Read the model definition and answer for the solid it produces. Units are mm, in the model's axes. A direction names the side the tool comes from. Give positions to 0.01 mm unless a question says otherwise; leave off trailing zeros. Order: outer loops, then holes, each group sorted by start corner. A loop starts at its lowest first (then second) coordinate and runs counter-clockwise, first axis right, second up. Notation, with made-up numbers: (8.25, -31.5) -> (23.25, -31.5) arc R24 ccw to (23.25, -2.5) -> close; hole circle Ø6 at (-0.5, -34). An arc over 180 degrees is marked (long way). One line per question, with ' | ' between items. Start each with the question number.
```python
from build123d import *

# Parameters (mm, degrees)
SKETCH1_R           = 10
BOSS_EXTRUDE1_DEPTH = 11
CUT_EXTRUDE1_DEPTH  = 2.5
CUT_EXTRUDE2_DEPTH  = 2.5
SKETCH4_W           = 15.449608091
SKETCH4_H           = 8
CUT_EXTRUDE3_DEPTH  = 3
FILLET1_R           = 1
CUT_EXTRUDE5_START  = -1.5
CUT_EXTRUDE5_DEPTH  = 1.5


with BuildPart() as part:
    # Sketch1 → Boss-Extrude1 (new, symmetric)
    with BuildSketch(Plane.XY):
        with BuildLine():
            ThreePointArc((16.711932938, -6.452050085), (11, 0), (16.711932938, 6.452050085))
            ThreePointArc((16.711932938, 6.452050085), (0, 36), (-16.711932938, 6.452050085))
            ThreePointArc((-16.711932938, 6.452050085), (-11, 0), (-16.711932938, -6.452050085))
            ThreePointArc((-16.711932938, -6.452050085), (0, -36), (16.711932938, -6.452050085))
        make_face()
        with Locations((0, -16.5)):
            Circle(SKETCH1_R, mode=Mode.SUBTRACT)
        with Locations((0, 16.5)):
            Circle(SKETCH1_R, mode=Mode.SUBTRACT)
    extrude(amount=BOSS_EXTRUDE1_DEPTH, both=True)

    # Sketch2 → Cut-Extrude1 (cut)
    with BuildSketch(Plane.XY.offset(11)):
        with BuildLine():
            Line((-19.068213964, 20.580835235), (-15.186057607, 18.339471217))
            ThreePointArc((-15.186057607, 18.339471217), (-13.000189211, 18.186313351), (-11.533289054, 19.814097705))
            ThreePointArc((-11.533289054, 19.814097705), (9.5856448, 23.719100621), (0, 4.5))
            ThreePointArc((0, 4.5), (-4.5, 0), (0, -4.5))
            ThreePointArc((0, -4.5), (9.5856448, -23.719100621), (-11.533289054, -19.814097705))
            ThreePointArc((-11.533289054, -19.814097705), (-13.000189211, -18.186313351), (-15.186057607, -18.339471217))
            Line((-15.186057607, -18.339471217), (-19.068213964, -20.580835235))
            ThreePointArc((-19.068213964, -20.580835235), (-18.199948236, -23.500848821), (-16.887495374, -26.25))
            Line((-16.887495374, -26.25), (-14.696938457, -24.985281374))
            ThreePointArc((-14.696938457, -24.985281374), (-13.966653368, -24.87818357), (-13.36182443, -25.301229909))
            ThreePointArc((-13.36182443, -25.301229909), (14.085802756, -24.088818138), (0, -0.5))
            ThreePointArc((0, -0.5), (-0.5, 0), (0, 0.5))
            ThreePointArc((0, 0.5), (14.085802756, 24.088818138), (-13.36182443, 25.301229909))
            ThreePointArc((-13.36182443, 25.301229909), (-13.966653368, 24.87818357), (-14.696938457, 24.985281374))
            Line((-14.696938457, 24.985281374), (-16.887495374, 26.25))
            ThreePointArc((-16.887495374, 26.25), (-18.199948236, 23.500848821), (-19.068213964, 20.580835235))
        make_face()
    extrude(amount=-CUT_EXTRUDE1_DEPTH, mode=Mode.SUBTRACT)

    # Sketch3 → Cut-Extrude2 (cut)
    with BuildSketch(Plane.XY.offset(11)):
        Polygon((-17.173443463, 0.521044654), (1.285575219, -14.967911114), (-1.285575219, -18.032088886), (-19.744593902, -2.543133118), align=None)
    cut_extrude2 = extrude(amount=-CUT_EXTRUDE2_DEPTH, mode=Mode.SUBTRACT)

    # Mirror1: Cut-Extrude2 across plane
    add(cut_extrude2.mirror(Plane.ZX), mode=Mode.SUBTRACT)

    # Sketch4 → Cut-Extrude3 (cut)
    with BuildSketch(Plane(origin=(0, 0, -11), x_dir=(-1, 0, 0), z_dir=(0, 0, -1))):
        with Locations((11.224804046, 0)):
            Rectangle(SKETCH4_W, SKETCH4_H)
        with Locations((-11.224804046, 0)):
            Rectangle(SKETCH4_W, SKETCH4_H)
    extrude(amount=-CUT_EXTRUDE3_DEPTH, mode=Mode.SUBTRACT)

    # Fillet1
    fillet1_edges = [part.edges().sort_by_distance(p)[0] for p in [
        (-3.5, 4, -9.5),
        (-3.5, -4, -9.5),
        (3.5, -4, -9.5),
        (3.5, 4, -9.5),
    ]]
    fillet(fillet1_edges, radius=FILLET1_R)

    # Sketch5 → Cut-Extrude5 (cut)
    with BuildSketch(Plane(origin=(0, 0, -11), x_dir=(-1, 0, 0), z_dir=(0, 0, -1)).offset(CUT_EXTRUDE5_START)):
        with BuildLine():
            ThreePointArc((12.376524617, 4), (13.243803843, 4.912717605), (14.270776222, 5.641109269))
            Line((14.270776222, 5.641109269), (7.397387325, 9.771057976))
            ThreePointArc((7.397387325, 9.771057976), (5.606135542, 8.219224415), (3.5, 7.132503002))
            Line((3.5, 7.132503002), (3.5, 3))
            ThreePointArc((3.5, 3), (3.792893219, 3.707106781), (4.5, 4))
            Line((4.5, 4), (12.376524617, 4))
        make_face()
        with BuildLine():
            Line((7.397387325, -9.771057976), (14.270776222, -5.641109269))
            ThreePointArc((14.270776222, -5.641109269), (13.243803843, -4.912717605), (12.376524617, -4))
            Line((12.376524617, -4), (4.5, -4))
            ThreePointArc((4.5, -4), (3.792893219, -3.707106781), (3.5, -3))
            Line((3.5, -3), (3.5, -7.132503002))
            ThreePointArc((3.5, -7.132503002), (5.606135542, -8.219224415), (7.397387325, -9.771057976))
        make_face()
    extrude(amount=CUT_EXTRUDE5_DEPTH, mode=Mode.SUBTRACT)


solid = part.part
```
Q1. A cutting plane is placed at B-B, the plane x = 8. Give the number of separate pieces and of enclosed holes in the cut face, then the cut area to 3 significant figures.
Q2. Which of the six approach directions +Z, -Z, +X, -X, +Y, -Y give full straight-line access (tool end or side, diameter ignored) to faces 1 (the flat face through (-15.81, -25.63, 9.77)), 2 (the flat face through (-17.1, -19.444, 9.768)), 3 (the flat face through (-10.88, 7.68, -10.24)), 4 (the flat face through (8, -4, -10)), 5 (the flat face through (-8, 4, -9))?
Q3. A cutting plane is placed at A-A, the plane y = -16.5. Determine the outline of the cut face in (x, z).
Q4. Given P1, Ø4, axis at x = 9.5, y = -1.5, coming from the -Z side; P2, Ø1.6, axis at x = -8.5, z = -8.5, coming from the -Y side; P3, Ø8, axis at y = 9, z = -5.5, coming from the -X side; P4, Ø18, axis at x = 0, y = -16.5, coming from the -Z side, each flat-ended and moving along its own axis, determine where each tip first touches the part or whether it passes through.
Q5. A cutting plane is placed at C-C, the plane z = 1.5. Determine the outline of the cut face in (x, y), then the cut area to 3 significant figures.
Q6. A cutting plane is placed at D-D, the plane x = 15. Determine the outline of the cut face in (y, z).
Q7. Find the intervals of material crossed by line 1 (X direction, y = -16.5, z = 9.95); line 2 (Y direction, x = 0, z = 2.75); line 3 (X direction, y = 17, z = 7.75), in increasing order.
Q8. Determine the mould class of faces 6 (the flat face through (-17.2, 19.5, 9.8)), 7 (the flat face through (-15.78, 25.61, 9.77)), 8 (the flat face through (-12.06, 8.99, 9.77)), 9 (the flat face through (8, 0, -8)) for opening direction X: pulls with the +X half, pulls with the -X half, needs draft (parallel to the pull), parting line crosses it, or undercut.
Geometry results:
1) separate pieces: 3 | enclosed holes: 0 | area: 907 mm²
2) face 1: +Z, -X | face 2: +Z | face 3: -Z | face 4: -Z, +X | face 5: -Z, -X
3) outline: (-19.5, -11) -> (-10, -11) -> (-10, 11) -> (-19.5, 11) -> close; (10, -11) -> (19.5, -11) -> (19.5, 11) -> (16, 11) -> (16, 8.5) -> (12, 8.5) -> (12, 11) -> (10, 11) -> close
4) P1: z = -8 | P2: y = -34.42 | P3: x = -19.18 | P4: through
5) outline: (-16.71, -6.45) arc R19.5 ccw (long way) to (16.71, -6.45) arc R6.5 cw to (16.71, 6.45) arc R19.5 ccw (long way) to (-16.71, 6.45) arc R6.5 cw to start; hole circle Ø20 at (0, -16.5); hole circle Ø20 at (0, 16.5) | area: 1,630 mm²
6) outline: (-28.96, -11) -> (-6, -11) -> (-6, 11) -> (-10.93, 11) -> (-10.93, 8.5) -> (-22.07, 8.5) -> (-22.07, 11) -> (-28.96, 11) -> close; (6, -11) -> (28.96, -11) -> (28.96, 11) -> (22.07, 11) -> (22.07, 8.5) -> (10.93, 8.5) -> (10.93, 11) -> (6, 11) -> close
7) line 1: -19.5 to -10, 10 to 12, 16 to 19.5 | line 2: -36 to -26.5, -6.5 to 6.5, 26.5 to 36 | line 3: -19.49 to -9.99, 9.99 to 19.49
8) face 6: undercut | face 7: pulls with the -X half | face 8: undercut | face 9: needs draft
